Input: part model. Units: mm. Frame: model coordinates. A direction names the side the tool comes from. Give positions to 0.01 mm unless a question says otherwise; leave off trailing zeros. Loops run counter-clockwise (first coordinate to the right, second up) from the corner with the lowest first, then second, coordinate; pieces in that order, holes last. Notation, with made-up numbers: M 88.25,69.25 L 119.25,69.25 A23 cw 119.25,99.25 Z; hole C -20.75,-30 d5. An arc over 180 degrees is marked long. Use CSV: the item, a comma, the result in double quotes. Start each with the question number.
Q1. Section B-B, the plane x = 33.5. Output: boundary loops of the cut face in (y, z).
Q2. Section A-A, the plane x = 7. Output: boundary loops of the cut face in (y, z), plus the area to 3 significant figures.
Q3. Pin query (flat end, axial travel): pin 1 (12 mm diameter, centred on x = 51.5, y = -0.5, fed in from -Z); pin 2 (4 mm diameter, centred on x = 11.5, z = -2.5, fed in from -Y); pin 3 (10 mm diameter, centred on x = 25, y = 8.5, fed in from -Z). Return the tip coordinate at first contact, or that it passes through.
Q4. Reachability of faces 1 (the flat face through (8.2, -9.5, 3.2)), 2 (the flat face through (0, 0, 0)) from +Z, -Z, +X, -X, +Y, -Y: full face, straight path, thin tool, end or side. Return the list, or none.
Q5. Material intervals for line 1 along X through (y, z) = (8.25, -4.25); line 2 along Y through (x, z) = (7.5, 1.5); line 3 along Y through (x, z) = (54.5, -0.25), sorted ascending.
from build123d import *

# Parameters (mm, degrees)
BOSS_EXTRUDE_DEPTH = 8.8
CHAMFER_2_SIZE     = 1.6


with BuildPart() as part:
    # Sketch1 → Boss-Extrude (new body)
    with BuildSketch(Plane(origin=(0, 0, 0), x_dir=(0, 0, -1), z_dir=(1, 0, 0))):
        Polygon((10.5, 6.062177826), (10.5, -6.062177826), (0, -12.124355653), (-10.5, -6.062177826), (-10.5, 6.062177826), (0, 12.124355653), align=None)
    extrude(amount=BOSS_EXTRUDE_DEPTH)

    # Sketch2 → Boss-Revolve1 (revolve)
    with BuildSketch(Plane.XY, mode=Mode.PRIVATE) as boss_revolve1_sk:
        Polygon((0, 0), (68.8, 0), (68.8, 5.268), (68.8, 7), (8.8, 7), (0, 7), align=None)
    revolve(boss_revolve1_sk.sketch.rotate(Axis((0, 0, 0), (-1, 0, 0)), 90), axis=Axis((0, 0, 0), (-1, 0, 0)))

    # Sketch3 → Cut-Revolve1 (revolve, cut)
    with BuildSketch(Plane.XY):
        Polygon((0, 10.5), (3.824573519, 17.124355653), (3.824573519, 22.124355653), (-10, 22.124355653), (-10, 10.5), align=None)
    revolve(axis=Axis((0, 0, 0), (1, 0, 0)), mode=Mode.SUBTRACT)

    # Sketch5 → Cut-Revolve2 (revolve, cut)
    with BuildSketch(Plane.XY):
        Polygon((8.8, 10.5), (4.975426481, 17.124355653), (4.975426481, 22.124355653), (14.975426481, 22.124355653), (14.975426481, 10.5), align=None)
    revolve(axis=Axis((0, 0, 0), (1, 0, 0)), mode=Mode.SUBTRACT)

    # Sketch4 → Cut-Revolve3 (revolve, cut)
    with BuildSketch(Plane.XY, mode=Mode.PRIVATE) as cut_revolve3_sk:
        Polygon((8.8, 9.517264973), (8.2, 9.863675135), (8.2, 22.124355653), (8.8, 22.124355653), align=None)
    revolve(cut_revolve3_sk.sketch.rotate(Axis((0, 0, 0), (1, 0, 0)), 90), axis=Axis((0, 0, 0), (1, 0, 0)), mode=Mode.SUBTRACT)

    # Chamfer 2
    chamfer_2_edges = [part.edges().sort_by_distance(p)[0] for p in [
        (68.8, 0, 7),
    ]]
    chamfer(chamfer_2_edges, length=CHAMFER_2_SIZE)

    # Sketch9 → Revolve1 (revolve)
    with BuildSketch(Plane.XY, mode=Mode.PRIVATE) as revolve1_sk:
        with BuildLine():
            Line((8.8, 7.6), (8.8, 7))
            Line((8.8, 7), (9.4, 7))
            ThreePointArc((9.4, 7), (8.975735931, 7.175735931), (8.8, 7.6))
        make_face()
    revolve(revolve1_sk.sketch.rotate(Axis((0, 0, 0), (1, 0, 0)), 90), axis=Axis((0, 0, 0), (1, 0, 0)))


solid = part.part
A:
1,outline,"C 0,0 d14"
2,outline,"M -12.12,0 L -6.06,-10.5 L 6.06,-10.5 L 12.12,0 L 6.06,10.5 L -6.06,10.5 Z"
2,area,"382 mm^2"
3,pin 1,"z = -7"
3,pin 2,"y = -6.98"
3,pin 3,"z = -6.06"
4,face 1,"+X"
4,face 2,"+Z, -Z, -X, +Y, -Y"
5,line 1,"0 to 8.8"
5,line 2,"-11.26 to 11.26"
5,line 3,"-7 to 7"
